from build123d import *

# Parameters (mm, degrees)
WALL_PLATE_DEPTH           = 6
LOWER_FLANGE_SKETCH_R      = 22
LOWER_FLANGE_44_DEPTH      = 6
PIVOT_BOSS_SKETCH_R        = 17
PIVOT_BOSS_34_DEPTH        = 70
UPPER_FLANGE_SKETCH_R      = 22
UPPER_FLANGE_DEPTH         = 6
PIVOT_BORE_SKETCH_R        = 8
PIVOT_BORE_16_DEPTH        = 173.580416038
SUPPORT_ARM_DEPTH          = 6
ARM_WEB_REACH              = 159.797
ARM_WEB_SKETCH_W           = 6
ARM_WEB_SKETCH_H           = 35
MOUNTING_HOLES_SKETCH_R    = 6
MOUNTING_HOLES_3X_12_DEPTH = 6
GUSSET_RIB_REACH           = 159.797
GUSSET_RIB_SKETCH_W        = 6
GUSSET_RIB_SKETCH_H        = 39


with BuildPart() as part:
    # Wall Plate Sketch → Wall Plate (new body)
    with BuildSketch(Plane.XY):
        with BuildLine():
            Line((-38, 64), (-15.192006216, -5.020253691))
            ThreePointArc((-15.192006216, -5.020253691), (0, -16), (15.192006216, -5.020253691))
            Line((15.192006216, -5.020253691), (38, 64))
            Line((38, 64), (38, 100))
            Line((38, 100), (-38, 100))
            Line((-38, 100), (-38, 64))
        make_face()
    extrude(amount=WALL_PLATE_DEPTH)



with BuildPart() as body_2:
    # Lower Flange Sketch → Lower Flange Ø44 (new body)
    with BuildSketch(Plane(origin=(0, 100, 0), x_dir=(1, 0, 0), z_dir=(0, 1, 0))):
        with Locations(Location((0, -100, 0), (0, 0, 180))):
            Circle(LOWER_FLANGE_SKETCH_R)
    extrude(amount=-LOWER_FLANGE_44_DEPTH)

    # Pivot Boss Sketch → Pivot Boss Ø34 (add)
    with BuildSketch(Plane.XZ.offset(-94)):
        with Locations((0, 100)):
            Circle(PIVOT_BOSS_SKETCH_R)
    extrude(amount=PIVOT_BOSS_34_DEPTH)

    # Upper Flange Sketch → Upper Flange (add)
    with BuildSketch(Plane.XZ.offset(-24)):
        with Locations(Location((0, 100, 0), (0, 0, 180))):
            Circle(UPPER_FLANGE_SKETCH_R)
    extrude(amount=UPPER_FLANGE_DEPTH)

    # Pivot Bore Sketch → Pivot Bore Ø16 (cut, through all)
    with BuildSketch(Plane(origin=(0, 100, 0), x_dir=(1, 0, 0), z_dir=(0, 1, 0))):
        with Locations(Location((0, -100, 0), (0, 0, 180))):
            Circle(PIVOT_BORE_SKETCH_R)
    extrude(amount=-PIVOT_BORE_16_DEPTH, mode=Mode.SUBTRACT)


with BuildPart() as part_1:
    add(part.part)

    add(body_2.part)  # Support Arm merges body 2
    # Support Arm Sketch → Support Arm (add)
    with BuildSketch(Plane(origin=(0, 65, 0), x_dir=(1, 0, 0), z_dir=(0, 1, 0))):
        with BuildLine():
            Line((-28, -6), (28, -6))
            Line((28, -6), (16.887127656, -101.955740153))
            ThreePointArc((16.887127656, -101.955740153), (0, -83), (-16.887127656, -101.955740153))
            Line((-16.887127656, -101.955740153), (-28, -6))
        make_face()
    extrude(amount=-SUPPORT_ARM_DEPTH)

    # Arm Web Sketch → Arm Web (add, up to next)
    with BuildSketch(Plane.XY.offset(6), mode=Mode.PRIVATE) as arm_web_sk1:
        with Locations((0, 82.5)):
            Rectangle(ARM_WEB_SKETCH_W, ARM_WEB_SKETCH_H)
    arm_web_tool1 = extrude(arm_web_sk1.sketch, amount=ARM_WEB_REACH, mode=Mode.PRIVATE) - part_1.part
    add(arm_web_tool1.solids().sort_by_distance((0, 82.5, 6))[0])

    # Mounting Holes Sketch → Mounting Holes 3xØ12 (cut)
    with BuildSketch(Plane.XY.offset(6)):
        Circle(MOUNTING_HOLES_SKETCH_R)
        with Locations((-22, 82)):
            Circle(MOUNTING_HOLES_SKETCH_R)
        with Locations((22, 82)):
            Circle(MOUNTING_HOLES_SKETCH_R)
    extrude(amount=-MOUNTING_HOLES_3X_12_DEPTH, mode=Mode.SUBTRACT)

    # Gusset Rib Sketch → Gusset Rib (add, up to next)
    with BuildSketch(Plane.XY.offset(6), mode=Mode.PRIVATE) as gusset_rib_sk1:
        with Locations((0, 39.5)):
            Rectangle(GUSSET_RIB_SKETCH_W, GUSSET_RIB_SKETCH_H)
    gusset_rib_tool1 = extrude(gusset_rib_sk1.sketch, amount=GUSSET_RIB_REACH, mode=Mode.PRIVATE) - part_1.part
    add(gusset_rib_tool1.solids().sort_by_distance((0, 39.5, 6))[0])


solid = part_1.part
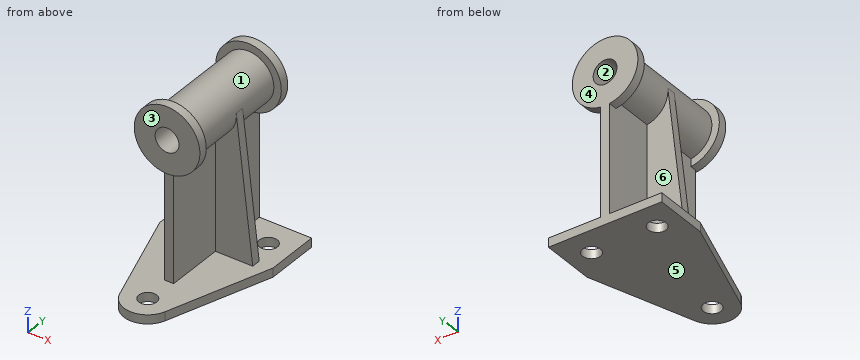
Can you work these out from the model? Positions are in its coordinate system, mm. Face numbers are marked on the shaded views. A direction names the side the tool comes from. Round coordinates to 2 decimals unless told otherwise and drop trailing zeros. Write each loop counter-clockwise with the first axis right and the second up, starting at its lowest first coordinate (ties: lowest second). Pieces come first, ordered by that corner, then holes. Notation, with made-up numbers: (86.5, 80) -> (112.5, 80) arc R28 cw to (112.5, 105) -> close; hole circle Ø2 at (49.5, 9.25). An arc over 180 degrees is marked (long way). One line per question, with ' | ' between items. Start each with the question number.
1) If we mould it in two halves opening along Z, with no side actions, what happens to the marked faces 4, 5 and 6? For each: released by +Z, released by -Z, zero draft, split by the parting line, or undercut.
2) Suppose I cut it at A-A on y = 82. Write out the boundary of the cut face in (x, z), then the cut area to 3 significant figures.
3) I'm going to push flat-ended pins straight in: P1, Ø1.5, axis at x = -6, y = 7, coming from the +Z side; P2, Ø8, axis at y = 75, z = 22.5, coming from the -X side; P3, Ø12.5, axis at x = -14.5, z = 64.5, coming from the -Y side. Where does each tip first touch, or does it pass through?
4) On a 3-axis mill with a long thin cutter (end or side, diameter ignored), from which of +Z, -Z, +X, -X, +Y, -Y can I reach the whole of each face in a straight line? I mean the marked faces 1, 2 and 3. Say none if no direction works.
5) Suppose I cut it at B-B on x = 0. Write out the boundary of the cut face in (y, z).
6) Suppose I cut it at D-D on x = 23.5. Write out the boundary of the cut face in (y, z).
7) Suppose I cut it at C-C on y = 22. Write out the boundary of the cut face in (x, z), then the cut area to 3 significant figures.
8) I need wall thicknesses on line 1 (Z direction, x = 5, y = 85) (3 decimals); line 2 (X direction, y = 38.5, z = 24); line 3 (Z direction, x = -10, y = 73.5). Which ranges of each line are inside material? Lowest first, please. Write a range as [from, to].
Return value:
1) face 4: zero draft | face 5: released by -Z | face 6: undercut
2) outline: (-38, 0) -> (-28, 0) -> (-28, 6) -> (-38, 6) -> close; (-16, 0) -> (16, 0) -> (16, 6) -> (3, 6) -> (3, 83.27) arc R17 ccw (long way) to (-3, 83.27) -> (-3, 6) -> (-16, 6) -> close; (28, 0) -> (38, 0) -> (38, 6) -> (28, 6) -> close; hole circle Ø16 at (0, 100) | area: 1,480 mm2
3) P1: stops at z = 6 | P2: stops at x = -3 | P3: stops at y = 59
4) face 1: none | face 2: +Y, -Y | face 3: +Z, +X, -X, -Y
5) outline: (-16, 0) -> (-6, 0) -> (-6, 6) -> (-16, 6) -> close; (6, 0) -> (100, 0) -> (100, 92) -> (18, 92) -> (18, 78) -> (20, 78) -> (20, 6) -> (6, 6) -> close; (18, 108) -> (100, 108) -> (100, 122) -> (94, 122) -> (94, 117) -> (24, 117) -> (24, 122) -> (18, 122) -> close
6) outline: (20.12, 0) -> (76.19, 0) -> (76.19, 6) -> (65, 6) -> (65, 44.86) -> (59, 44.86) -> (59, 6) -> (20.12, 6) -> close; (87.81, 0) -> (100, 0) -> (100, 6) -> (87.81, 6) -> close
7) outline: (-24.12, 0) -> (24.12, 0) -> (24.12, 6) -> (3, 6) -> (3, 78.21) arc R22 ccw (long way) to (-3, 78.21) -> (-3, 6) -> (-24.12, 6) -> close; hole circle Ø16 at (0, 100) | area: 2,040 mm2
8) line 1: z = [0, 6], [83.752, 93.755], [106.245, 116.248] | line 2: x = [-3, 3] | line 3: z = [0, 6], [86.25, 113.75]
